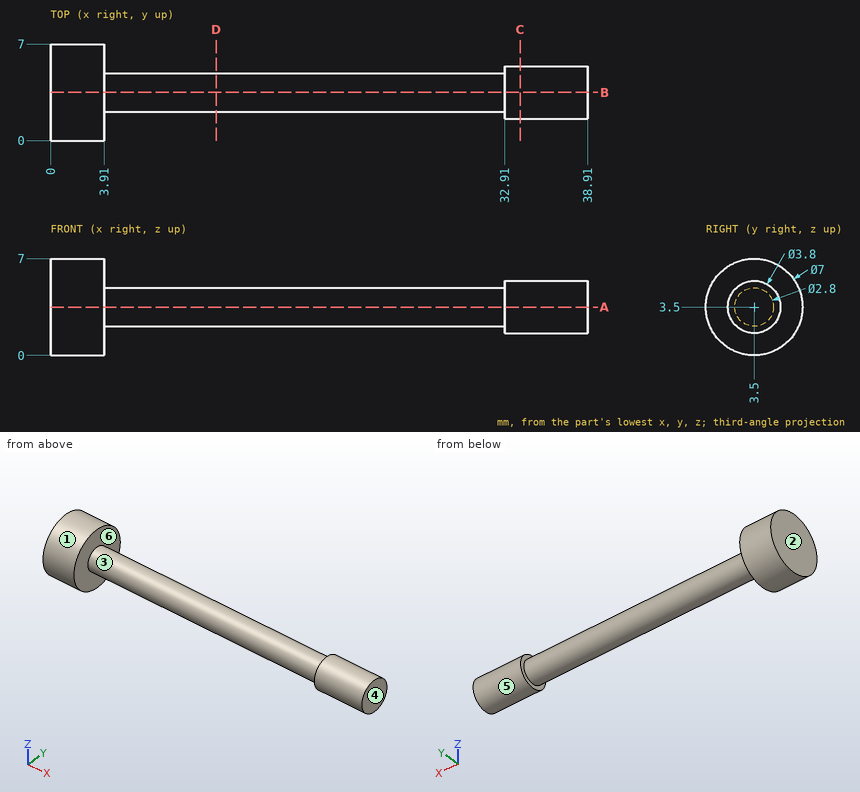
Answer from the drawing. Dimensions are ordinates in mm from the lowest x, y and z of the part. A direction names the side the tool comes from. Round coordinates to 2 decimals unless told otherwise and drop trailing zeros. Loops run counter-clockwise (first coordinate to the right, second up) from the corner with the lowest first, then second, coordinate; pieces in that order, holes last.
(1) The part is cut by section A-A, the plane z = 3.5. Give the vertices of the cut face in (x, y), and give its area (3 significant figures).
Computed values:
outline: (0, 0) - (3.91, 0) - (3.91, 2.1) - (32.91, 2.1) - (32.91, 1.6) - (38.91, 1.6) - (38.91, 5.4) - (32.91, 5.4) - (32.91, 4.9) - (3.91, 4.9) - (3.91, 7) - (0, 7) - close
area: 131 mm2
(2) The mould has two halves that part along X. Classify the marked faces 1, 2, 3 and 4: pulls with the +X half, pulls with the -X half, needs draft (parallel to the pull), parting line crosses it, or undercut.
Computed values:
face 1: needs draft
face 2: pulls with the -X half
face 3: undercut
face 4: pulls with the +X half
(3) The part is cut by section C-C, the plane x = 34. Give the vertices of the cut face in (y, z).
Computed values:
outline: circle Ø3.8 at (3.5, 3.5)
(4) Find the intervals of material crossed by L1, parallel to X at y = 2.75, z = 5; L2, parallel to Y at x = 23, z = 3.5; L3, parallel to X at y = 5.25, z = 0.5, in increasing order.
Computed values:
L1: x = 0 to 3.91, 32.91 to 38.91
L2: y = 2.1 to 4.9
L3: x = 0 to 3.91
(5) The part is cut by section D-D, the plane x = 12. Give the vertices of the cut face in (y, z), and give its area (3 significant figures).
Computed values:
outline: circle Ø2.8 at (3.5, 3.5)
area: 6.16 mm2
(6) Each of these flat-tipped pins is pushed along its axis until it touches: P1, Ø1, axis at x = 29.5, y = 2.5, coming from the +Z side; P2, Ø4, axis at y = 4, z = 3, coming from the -X side; P3, Ø4, axis at x = 16.5, y = 6, coming from the -Z side; P4, Ø2, axis at x = 15, y = 3.5, coming from the +Z side. Where does it stop, or does it pass through?
Computed values:
P1: stops at z = 4.81
P2: stops at x = 0
P3: stops at z = 2.19
P4: stops at z = 4.9
(7) For the marked faces 5 and 6, determine the directions among +Z, -Z, +X, -X, +Y, -Y from which every point of the face is accessible in a straight line to the end or side of a thin tool.
Computed values:
face 5: +X
face 6: none
